Answer from the drawing. Dimensions are ordinates in mm from the lowest x, y and z of the part. A direction names the side the tool comes from. Coordinates: 2 decimals unless noted, no trailing zeros. Write each loop counter-clockwise with the first axis right and the second up, starting at its lowest first coordinate (ties: lowest second). Pieces come first, ordered by that corner, then holes.
(1) Straight lines are drawn through the part: line 1 along X through (y, z) = (10.5, 30); line 2 along X through (y, z) = (28, 30); line 3 along Z through (x, y) = (38.5, 19). For each, find the intervals that lie inside material, in ascending order.
(2) Given pin 1 (18 mm diameter, centred on x = 22, z = 34, fed in from +Y); pin 2 (4 mm diameter, centred on y = 5, z = 52.5, fed in from +X); pin 3 (5 mm diameter, centred on y = 29, z = 52, fed in from +X), each flat-ended and moving along its own axis, determine where each tip first touches the part or whether it passes through.
(3) Which of the six approach directions +Z, -Z, +X, -X, +Y, -Y give full straight-line access (tool end or side, diameter ignored) to the marked faces 1 and 2?
(4) Determine the mould class of the marked faces 3, 4 and 5 for opening direction Z: pulls with the +Z half, pulls with the -Z half, needs draft (parallel to the pull), parting line crosses it, or undercut.
(5) The part is cut by section D-D, the plane x = 51.5. Determine the outline of the cut face in (y, z), and give its area (3 significant figures).
(6) The part is cut by section C-C, the plane y = 10. Determine the outline of the cut face in (x, z).
(7) The part is cut by section B-B, the plane x = 30. Determine the outline of the cut face in (y, z).
(8) The part is cut by section A-A, the plane z = 30. Determine the outline of the cut face in (x, y).
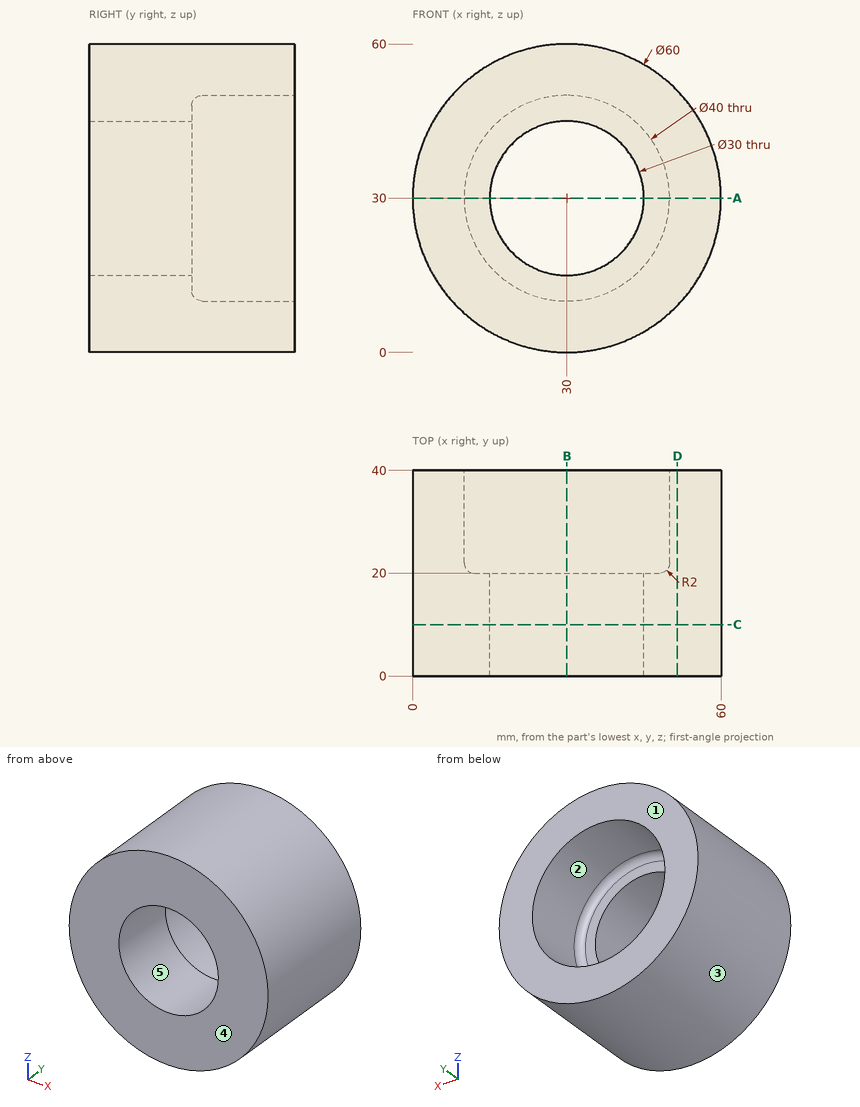
Computed:
1. line 1: x = 0 to 15, 45 to 60
1. line 2: x = 0 to 10, 50 to 60
1. line 3: z = 1.23 to 17.64, 42.36 to 58.77
2. pin 1: stops at y = 20
2. pin 2: stops at x = 51.9
2. pin 3: stops at x = 52.8
3. face 1: +Z, -Z, +X, -X, +Y
3. face 2: +Y
4. face 3: parting line crosses it
4. face 4: needs draft
4. face 5: undercut
5. outline: (0, 9.08) - (40, 9.08) - (40, 50.92) - (0, 50.92) - close
5. area: 1,670 mm2
6. outline: circle Ø60 at (30, 30); hole circle Ø30 at (30, 30)
7. outline: (0, 0) - (40, 0) - (40, 10) - (22, 10) arc R2 cw to (20, 12) - (20, 15) - (0, 15) - close; (0, 45) - (20, 45) - (20, 48) arc R2 cw to (22, 50) - (40, 50) - (40, 60) - (0, 60) - close
8. outline: (0, 0) - (15, 0) - (15, 20) - (12, 20) arc R2 cw to (10, 22) - (10, 40) - (0, 40) - close; (45, 0) - (60, 0) - (60, 40) - (50, 40) - (50, 22) arc R2 cw to (48, 20) - (45, 20) - close
